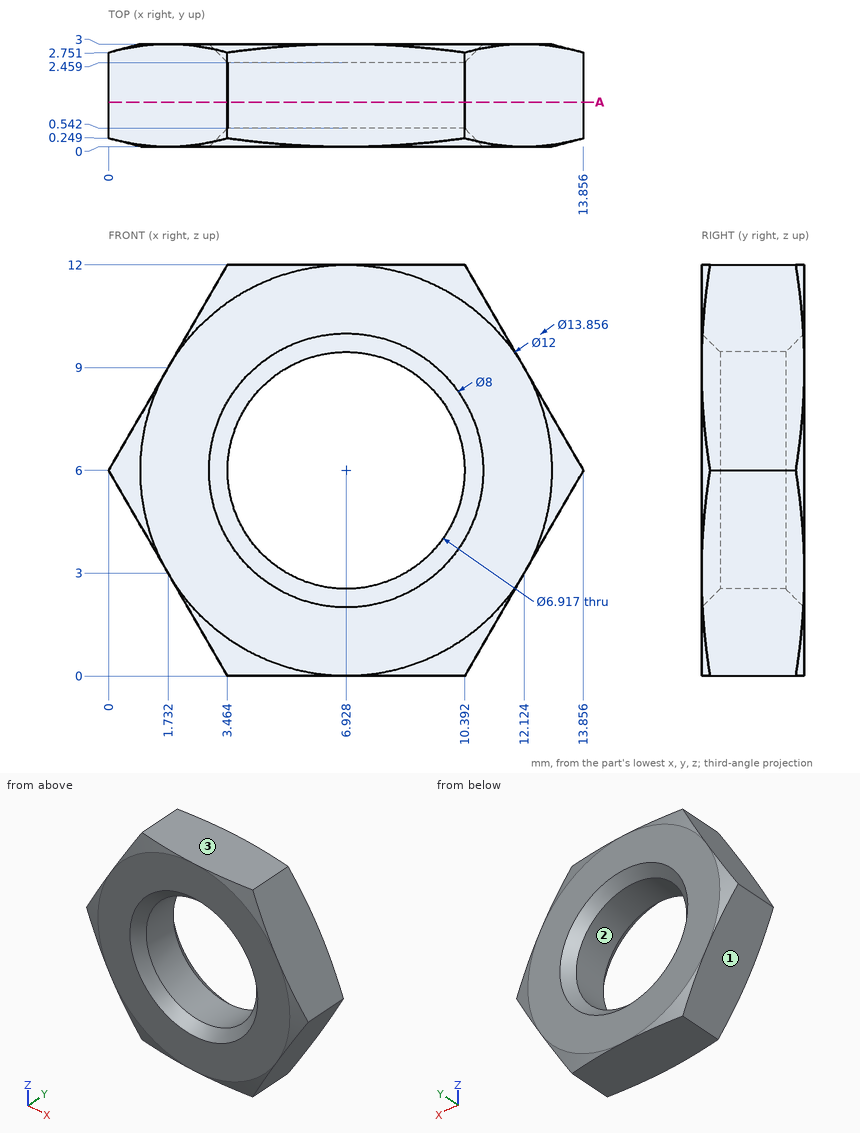
Verification items for this drawing (mm, ordinates from the low corner). Give positions to 0.01 mm unless a question says otherwise; leave off trailing zeros. Loops run counter-clockwise (first coordinate to the right, second up) from the corner with the lowest first, then second, coordinate; pieces in that order, holes last. Notation, with made-up numbers: (6, -12) - (64, -12) arc R23 cw to (64, -3) - close; hole circle Ø5 at (-13, 1.5). An arc over 180 degrees is marked (long way). Write item = value, one per line. Start each with the question number.
Q1. Depth check by flat-ended pin: P1, Ø6, axis at x = 6.93, z = 6, coming from the -Y side; P2, Ø1.5, axis at y = 2, z = 4.5, coming from the -X side. Enter the tip coordinate at first touch or a pass-through.
Q2. Thickness scan on line 1 (X direction, y = 1.55, z = 4.75) (1 decimal); line 2 (X direction, y = 1.3, z = 4.5) (1 decimal); line 3 (Z direction, x = 8.5, y = 0.5) (1 decimal). Record the ranges inside material, lowest first.
Q3. Mould release check, pull along X, two halves, no side actions. Record for the marked faces 1, 2 and 3: released by +X, released by -X, zero draft, split by the parting line, or undercut.
Q4. Cross-section at A-A, the plane y = 1.3. Enter the section's corners in (x, z) (1 decimal).
Answer key:
q1.P1 = through
q1.P2 = 0.43
q2.line_1 = 0.7 to 3.7, 10.2 to 13.1
q2.line_2 = 0.9 to 3.8, 10 to 13
q2.line_3 = 0 to 2.9, 9.1 to 12
q3.face_1 = released by -X
q3.face_2 = undercut
q3.face_3 = zero draft
q4.outline = (0, 6) - (3.5, 0) - (10.4, 0) - (13.9, 6) - (10.4, 12) - (3.5, 12) - close; hole circle Ø6.9 at (6.9, 6)
